from build123d import *

# Parameters (mm, degrees)
BOSS_EXTRUDE1_DEPTH          = 25
CUT_EXTRUDE1_REACH           = 1039.876
M16_TAPPED_HOLE1_D           = 14
M16_TAPPED_HOLE1_CSINK_D     = 16.05
M16_TAPPED_HOLE1_CSINK_ANGLE = 90
CIRPATTERN1_COUNT            = 12
M8_TAPPED_HOLE1_D            = 6.8
M8_TAPPED_HOLE1_CSINK_D      = 8.05
M8_TAPPED_HOLE1_CSINK_ANGLE  = 90
LPATTERN1_COUNT              = 3
LPATTERN1_PITCH              = 130
MIRROR1_COPY_1_D             = 6.8
MIRROR1_COPY_1_CSINK_D       = 8.05
MIRROR1_COPY_1_CSINK_ANGLE   = 90
MIRROR1_COPY_2_D             = 6.8
MIRROR1_COPY_2_CSINK_D       = 8.05
MIRROR1_COPY_2_CSINK_ANGLE   = 90
CHAMFER1_SIZE                = 5


with BuildPart() as part:
    # Sketch1 → Boss-Extrude1 (new body)
    with BuildSketch(Plane(origin=(0, 0, 0), x_dir=(0, 0, -1), z_dir=(1, 0, 0))):
        with BuildLine():
            Line((-387.5, 575), (-387.5, 0))
            Line((-387.5, 0), (387.5, 0))
            Line((387.5, 0), (387.5, 575))
            ThreePointArc((387.5, 575), (0, 962.5), (-387.5, 575))
        make_face()
    extrude(amount=BOSS_EXTRUDE1_DEPTH)

    # Sketch2 → Cut-Extrude1 (cut, up to next)
    with BuildSketch(Plane(origin=(25, 0, 0), x_dir=(0, 0, -1), z_dir=(1, 0, 0)), mode=Mode.PRIVATE) as cut_extrude1_sk1:
        with BuildLine():
            Line((-24.434111456, 672.999868354), (338.559277668, 763.504285109))
            ThreePointArc((338.559277668, 763.504285109), (375.065307711, 672.37692207), (387.5, 575))
            Line((387.5, 575), (387.5, 567.522624537))
            Line((387.5, 567.522624537), (24.434111456, 477.000131646))
            ThreePointArc((24.434111456, 477.000131646), (-97.999868354, 550.565888544), (-24.434111456, 672.999868354))
        make_face()
    cut_extrude1_tool1 = extrude(cut_extrude1_sk1.sketch, amount=-CUT_EXTRUDE1_REACH, mode=Mode.PRIVATE) & part.part
    add(cut_extrude1_tool1.solids().sort_by_distance((25, 611.611981, -146.843429))[0], mode=Mode.SUBTRACT)

    # M16 Tapped Hole1 (through all)
    with Locations(Plane(origin=(25, 696.286965784, 30.24023695), x_dir=(0, 0, 1), z_dir=(1, 0, 0))):
        with Locations((0, 0)):
            m16_tapped_hole1 = CounterSinkHole(M16_TAPPED_HOLE1_D / 2, M16_TAPPED_HOLE1_CSINK_D / 2, counter_sink_angle=M16_TAPPED_HOLE1_CSINK_ANGLE)

    # CirPattern1: M16 Tapped Hole1 ×12 about axis, 5 skipped
    cirpattern1_axis = Axis((-0.001, 575, 0), (-1, 0, 0))
    add([m16_tapped_hole1.rotate(cirpattern1_axis, i * 360 / CIRPATTERN1_COUNT) for i in range(1, CIRPATTERN1_COUNT) if i not in (1, 2, 3, 4, 5)], mode=Mode.SUBTRACT)

    # M8 Tapped Hole1 (through all)
    with Locations(Plane(origin=(25, 706.689607295, -11.48247928), x_dir=(0, 0, 1), z_dir=(1, 0, 0))):
        with Locations((0, 0)):
            m8_tapped_hole1 = CounterSinkHole(M8_TAPPED_HOLE1_D / 2, M8_TAPPED_HOLE1_CSINK_D / 2, counter_sink_angle=M8_TAPPED_HOLE1_CSINK_ANGLE)

    # LPattern1: M8 Tapped Hole1 ×3
    with Locations(*[Vector(0, 0.24192189559966076, -0.9702957262759982) * (i * LPATTERN1_PITCH) for i in range(1, LPATTERN1_COUNT)]):
        add(m8_tapped_hole1, mode=Mode.SUBTRACT)

    # Mirror1: M8 Tapped Hole1 across plane
    add(m8_tapped_hole1.mirror(Plane(origin=(0, 541.347432947, 134.973074301), x_dir=(0, -0.24192189559966135, 0.970295726275998), z_dir=(0, 0.9702957262759981, 0.24192189559966135))), mode=Mode.SUBTRACT)

    # Mirror1 copy 1 (through all)
    with Locations(Plane(origin=(25, 495.565522155, -198.101397596), x_dir=(0, -0.4694715627858792, 0.8829475928589331), z_dir=(1, 0, 0))):
        with Locations((0, 0)):
            CounterSinkHole(MIRROR1_COPY_1_D / 2, MIRROR1_COPY_1_CSINK_D / 2, counter_sink_angle=MIRROR1_COPY_1_CSINK_ANGLE)

    # Mirror1 copy 2 (through all)
    with Locations(Plane(origin=(25, 527.015368582, -324.239842012), x_dir=(0, -0.4694715627858792, 0.8829475928589331), z_dir=(1, 0, 0))):
        with Locations((0, 0)):
            CounterSinkHole(MIRROR1_COPY_2_D / 2, MIRROR1_COPY_2_CSINK_D / 2, counter_sink_angle=MIRROR1_COPY_2_CSINK_ANGLE)

    # Chamfer1
    chamfer1_edges = [part.edges().sort_by_distance(p)[0] for p in [
        (0, 950.065307711, 97.37692207),
        (25, 950.065307711, 97.37692207),
        (25, 283.761312269, -387.5),
        (0, 283.761312269, -387.5),
        (0, 287.5, 387.5),
        (25, 287.5, 387.5),
    ]]
    chamfer(chamfer1_edges, length=CHAMFER1_SIZE)


solid = part.part
Verification items for the finished model (mm, model axes). A direction names the side the tool comes from. Coordinates: 2 decimals unless noted, no trailing zeros. Write each question's results on one line, items separated by ' | '.
1) Access from +Z, -Z, +X, -X, +Y, -Y to the whole of each face (thin tool, end or side, straight path). Record for faces 5 (the face through (12.67, 717.62, -154.52)), 6 (the face through (0, 379, 5)).
Solved:
face 5: -Z, +X, -X | face 6: +Z, -Z, -X, +Y, -Y
2) Release check for a two-part mould opening along Y. For faces 1 (the face through (0.313, 947.239, 89.352)), 2 (the face through (12, 0, 5)), 3 (the face through (12.68, 548.42, 97.44)), 4 (the face through (12.675, 522.895, -208.509)) record: pulls with the +Y half, pulls with the -Y half, needs draft (parallel to the pull), parting line crosses it, or undercut.
Solved:
face 1: pulls with the +Y half | face 2: pulls with the -Y half | face 3: undercut | face 4: undercut
3) Gauge pin test, flat ends, axial feed: pin 1 Ø8 at (y, z) = (738.14, -137.62) entering from -X; pin 2 Ø2 at (x, z) = (14, 218.5) entering from +Y; pin 3 Ø5.5 at (y, z) = (527.02, -324.24) entering from -X; pin 4 Ø1 at (x, y) = (12, 625) entering from -Z. Record the tip position at first contact, or that the pin passes through.
Solved:
pin 1: stops at x = 0 | pin 2: stops at y = 895.7 | pin 3: passes through | pin 4: stops at z = 87.47
4) Scan lines: line 1 along Y through (x, z) = (6, 48); line 2 along Y through (x, z) = (15.5, -6.5); line 3 along Z through (x, y) = (19.75, 772.5). Record each from-to range of solid material in increasing order. Write a range as [from, to].
Solved:
line 1: y = [0, 486.13], [663.87, 959.52] | line 2: y = [0, 474.21], [680.71, 962.45] | line 3: z = [-333.39, -265.52], [-262, 333.39]
5) Section check A-A on x = 11.25. Give the number of separate pieces and of enclosed holes in the cut face, plus the area to 3 significant figures.
Solved:
separate pieces: 1 | enclosed holes: 13 | area: 587,000 mm²
